Source: CAD feature listing. Evaluate the final solid. Frame: model axes, mm. A direction names the side the tool comes from. Coordinates: 2 decimals unless noted, no trailing zeros. Order: outer loops, then holes, each group sorted by start corner. A loop starts at its lowest first (then second) coordinate and runs counter-clockwise, first axis right, second up.
```python
from build123d import *

# Parameters (mm, degrees)
BASE_BLOCK_PROFILE_W       = 45
BASE_BLOCK_PROFILE_H       = 32
BASE_BLOCK_DEPTH           = 41
END_SLOT_PROFILE_W         = 12
END_SLOT_PROFILE_H         = 7
END_SLOT_7X12_DEPTH        = 45
ARM_EXTENSION_DEPTH        = 41
UNDERSIDE_RELIEF_PROFILE_R = 6
UNDERSIDE_RELIEF_CUT_DEPTH = 50
RAISED_START               = 5
RAISED_PAD_DEPTH           = 5
PIVOT_BORE_PROFILE_R       = 9
PIVOT_BORE_18_DEPTH        = 50
PAD_CHAMFER_3X45_A_SIZE    = 3
PAD_CHAMFER_3X45_B_SIZE    = 3


with BuildPart() as part:
    # Base Block Profile → Base Block (new body)
    with BuildSketch(Plane.XY):
        with Locations((22.5, -16)):
            Rectangle(BASE_BLOCK_PROFILE_W, BASE_BLOCK_PROFILE_H)
    extrude(amount=BASE_BLOCK_DEPTH)

    # End Slot Profile → End Slot 7x12 (cut)
    with BuildSketch(Plane(origin=(45, 0, 0), x_dir=(0, 0, -1), z_dir=(1, 0, 0))):
        with Locations((-20.5, -28.5)):
            Rectangle(END_SLOT_PROFILE_W, END_SLOT_PROFILE_H)
    extrude(amount=-END_SLOT_7X12_DEPTH, mode=Mode.SUBTRACT)

    # Arm Extension Profile → Arm Extension (add)
    with BuildSketch(Plane.XY.offset(41)):
        with BuildLine():
            Line((-15, 21), (-65, 21))
            ThreePointArc((-65, 21), (-86, 0), (-65, -21))
            Line((-65, -21), (-9.998816778, -21.84617205))
            ThreePointArc((-9.998816778, -21.84617205), (-9.844988828, -21.847355271), (-9.69119728, -21.850904657))
            ThreePointArc((-9.69119728, -21.850904657), (-2.873570133, -24.829701409), (0, -31.692344099))
            Line((0, -31.692344099), (0, -22))
            Line((0, -22), (0, 0))
            Line((0, 0), (-15, 21))
        make_face()
    extrude(amount=-ARM_EXTENSION_DEPTH)

    # Underside Relief Profile → Underside Relief Cut (cut)
    with BuildSketch(Plane(origin=(0, 21, 0), x_dir=(1, 0, 0), z_dir=(0, 1, 0))):
        with Locations(Location((-29, -20.5, 0), (0, 0, 270))):
            Circle(UNDERSIDE_RELIEF_PROFILE_R)
        with Locations(Location((21, -20.5, 0), (0, 0, 90))):
            Circle(UNDERSIDE_RELIEF_PROFILE_R)
    extrude(amount=-UNDERSIDE_RELIEF_CUT_DEPTH, mode=Mode.SUBTRACT)

    # Raised Pad Profile → Raised Pad (add)
    with BuildSketch(Plane.XY.offset(41).offset(RAISED_START)):
        with BuildLine():
            Line((-44, 21), (-44, 0))
            Line((-44, 0), (-44, -21.323076923))
            Line((-44, -21.323076923), (-9.998816778, -21.84617205))
            ThreePointArc((-9.998816778, -21.84617205), (-2.982346138, -24.720925405), (0, -31.692344099))
            ThreePointArc((0, -31.692344099), (0.001183222, -31.84617205), (0, -32))
            Line((0, -32), (45, -32))
            Line((45, -32), (45, 0))
            Line((45, 0), (0, 0))
            Line((0, 0), (-15, 21))
            Line((-15, 21), (-44, 21))
        make_face()
    extrude(amount=-RAISED_PAD_DEPTH)

    # Pivot Bore Profile → Pivot Bore Ø18 (cut)
    with BuildSketch(Plane.XY.offset(41)):
        with Locations((-65, 0)):
            Circle(PIVOT_BORE_PROFILE_R)
    extrude(amount=-PIVOT_BORE_18_DEPTH, mode=Mode.SUBTRACT)

    # Pad Chamfer 3x45 A
    pad_chamfer_3x45_a_edges = [part.edges().sort_by_distance(p)[0] for p in [
        (-29.5, 21, 46),
    ]]
    chamfer(pad_chamfer_3x45_a_edges, length=PAD_CHAMFER_3X45_A_SIZE)

    # Pad Chamfer 3x45 B
    pad_chamfer_3x45_b_edges = [part.edges().sort_by_distance(p)[0] for p in [
        (45, -16, 46),
    ]]
    chamfer(pad_chamfer_3x45_b_edges, length=PAD_CHAMFER_3X45_B_SIZE)


solid = part.part
```
1. Section query A-A on z = 17. Return loops of the section in (x, y), plus the area to 3 significant figures.
Findings:
outline: (-65, -21) - (-33.87, -21.48) - (-33.87, 21) - (-65, 21) arc R21 ccw to start; (-24.13, -21.63) - (-10, -21.85) arc R10 cw to (-9.69, -21.85) arc R10 cw to (0, -31.69) - (0, -25) - (16.13, -25) - (16.13, 0) - (0, 0) - (-15, 21) - (-24.13, 21) - close; (25.87, -25) - (45, -25) - (45, 0) - (25.87, 0) - close; hole circle Ø18 at (-65, 0)
area: 3,530 mm2
2. Access query for faces 1 (the face through (23, -29, 26.5)), 2 (the face through (-56, 5, 41)), 3 (the face through (28, 0, 23)). Directions: +Z, -Z, +X, -X, +Y, -Y. A direction counts if a zero-diameter tool reaches every point of the face in a straight line with its end or side. Return the directions, or none.
Findings:
face 1: +X, -Y
face 2: +Z, -X, +Y, -Y
face 3: +Z, -Z, +X, +Y
3. Section query C-C on x = 29.5. Return loops of the section in (y, z).
Findings:
outline: (-32, 0) - (0, 0) - (0, 46) - (-32, 46) - (-32, 26.5) - (-25, 26.5) - (-25, 14.5) - (-32, 14.5) - close
4. Draft query along Z for faces 4 (the face through (36, -25, 21)), 5 (the face through (22, -32, 7)), 6 (the face through (-21, -5, 0)). Return one class per face: released by +Z, released by -Z, zero draft, split by the parting line, or undercut.
Findings:
face 4: undercut
face 5: zero draft
face 6: released by -Z
5. Ray query, line 1 (Y direction, x = -64.5, z = 33.5); line 2 (X direction, y = -14, z = 19); line 3 (Z direction, x = 26, y = -28). Return the intervals inside material, ascending.
Findings:
line 1: y = -21.01 to -8.99, 8.99 to 21
line 2: x = -80.65 to -34.81, -23.19 to 15.19, 26.81 to 45
line 3: z = 0 to 14.5, 26.5 to 46
6. Pin query (flat end, axial travel): P1, Ø5.5, axis at y = -30, z = 17.5, coming from the +X side; P2, Ø1, axis at x = -18, z = 32, coming from the -Y side; P3, Ø5, axis at y = 5.5, z = 17, coming from the +X side; P4, Ø9.5, axis at x = 9, z = 18, coming from the -Y side. Return the tip coordinate at first contact, or that it passes through.
Findings:
P1: stops at x = 0
P2: stops at y = -21.73
P3: stops at x = -2.14
P4: stops at y = -32
7. Section query D-D on y = -19. Return loops of the section in (x, z).
Findings:
outline: (-73.94, 0) - (45, 0) - (45, 43) - (42, 46) - (-44, 46) - (-44, 41) - (-73.94, 41) - close; hole circle Ø12 at (-29, 20.5); hole circle Ø12 at (21, 20.5)
8. Section query B-B on y = 7. Return loops of the section in (x, z).
Findings:
outline: (-84.8, 0) - (-70.66, 0) - (-70.66, 41) - (-84.8, 41) - close; (-59.34, 0) - (-5, 0) - (-5, 46) - (-44, 46) - (-44, 41) - (-59.34, 41) - close; hole circle Ø12 at (-29, 20.5)
